from build123d import *

# Parameters (mm, degrees)
SKETCH1_R             = 162.5
SKETCH1_R_2           = 120
BOSS_EXTRUDE1_DEPTH   = 180
SKETCH2_R             = 135
CUT_EXTRUDE1_DEPTH    = 160
CHAMFER1_SIZE         = 1
CHAMFER1_SIZE2        = 3
CHAMFER2_SIZE         = 1
M8_TAPPED_HOLE1_D     = 6.8
M8_TAPPED_HOLE1_DEPTH = 26
M8_TAPPED_HOLE1_TIP   = 2.042926105


with BuildPart() as part:
    # Sketch1 → Boss-Extrude1 (new body)
    with BuildSketch(Plane(origin=(0, 0, 0), x_dir=(1, 0, 0), z_dir=(0, 1, 0))):
        with Locations(Location((0, 0, 0), (0, 0, 90))):
            Circle(SKETCH1_R)
        with Locations(Location((0, 0, 0), (0, 0, 90))):
            Circle(SKETCH1_R_2, mode=Mode.SUBTRACT)
    extrude(amount=BOSS_EXTRUDE1_DEPTH)

    # Sketch2 → Cut-Extrude1 (cut)
    with BuildSketch(Plane(origin=(0, 180, 0), x_dir=(1, 0, 0), z_dir=(0, 1, 0))):
        with Locations(Location((0, 0, 0), (0, 0, 270))):
            Circle(SKETCH2_R)
    extrude(amount=-CUT_EXTRUDE1_DEPTH, mode=Mode.SUBTRACT)

    # Chamfer1
    chamfer1_edges = [part.edges().sort_by_distance(p)[0] for p in [
        (0, 180, -135),
    ]]
    chamfer1_side = [part.faces().sort_by_distance(p)[0] for p in [
        (0, 180, 157.903805922),
    ]]
    chamfer(chamfer1_edges, length=CHAMFER1_SIZE, length2=CHAMFER1_SIZE2, reference=chamfer1_side[0])

    # Chamfer2
    chamfer2_edges = [part.edges().sort_by_distance(p)[0] for p in [
        (0, 20, 120),
        (0, 0, 120),
    ]]
    chamfer(chamfer2_edges, length=CHAMFER2_SIZE)

    # M8 Tapped Hole1
    with Locations(Plane(origin=(0, 180, 0), x_dir=(1, 0, 0), z_dir=(0, 1, 0))):
        with Locations((148, 0), (0, -148), (-148, 0), (0, 148)):
            Hole(M8_TAPPED_HOLE1_D / 2, depth=M8_TAPPED_HOLE1_DEPTH)
            with Locations((0, 0, -(M8_TAPPED_HOLE1_DEPTH + M8_TAPPED_HOLE1_TIP / 2))):  # 118° drill point
                Cone(0, M8_TAPPED_HOLE1_D / 2, M8_TAPPED_HOLE1_TIP, mode=Mode.SUBTRACT)


solid = part.part
Could you check a few things on this model? Use its own coordinates, in mm. A direction names the side the tool comes from. Coordinates: 2 decimals unless noted, no trailing zeros. Order: outer loops, then holes, each group sorted by start corner. A loop starts at its lowest first (then second) coordinate and runs counter-clockwise, first axis right, second up. Notation, with made-up numbers: (79, -1) -> (83, -1) arc R18 ccw to (83, 4) -> close; hole circle Ø10 at (-18, -36.75). An arc over 180 degrees is marked (long way). One line per item, written item: value. Start each with the question number.
1) We'd pull the mould along Z, two halves only. Please class faces 3 (the cylindrical face through (-137.02, 88.74, -87.36)), 4 (the cylindrical face through (-119.77, 99.6, 62.29)), 5 (the flat face through (84, 180, -108)): +Z half, -Z half, draft (parallel to the pull), parting line (faces both ways), or undercut.
2) If I drill on L1, parallel to X at y = 108, z = 0; L2, parallel to X at y = 153.5, z = 4.5; L3, parallel to Z at x = -148, y = 173, over which ranges is the centre line in solid material (lowest first)? Write a range as [from, to].
3) Which directions (+Z, -Z, +X, -X, +Y, -Y) give clear straight access to the entire face, cutting with the end or side of a thin tool? Please do faces 1 (the cylindrical face through (-5.276, 9.874, 119.884)), 2 (the flat face through (111, 20, -51)).
4) Imagine slicing it at B-B on y = 72.5. List the corners of the cut face in (x, z) for me, plus the area to 3 significant figures.
5) Imagine slicing it at A-A on y = 13.5. List the corners of the cut face in (x, z) for me, plus the area to 3 significant figures.
6) I'm going to push flat-ended pins straight in: pin 1 (6 mm diameter, centred on x = 104.5, y = 122.5, fed in from -Z); pin 2 (2 mm diameter, centred on y = 128, z = 70.5, fed in from -X); pin 3 (5 mm diameter, centred on x = -117.5, y = 42.5, fed in from -Z). Where does each tip first touch, or does it pass through?
Answer list:
1. face 3: parting line
1. face 4: undercut
1. face 5: draft
2. L1: x = [-162.5, -135], [135, 162.5]
2. L2: x = [-162.44, -134.92], [134.92, 162.44]
2. L3: z = [-67.1, -3.4], [3.4, 67.1]
3. face 1: +Y, -Y
3. face 2: +Y
4. outline: circle Ø325 at (0, 0); hole circle Ø270 at (0, 0)
4. area: 25,700 mm2
5. outline: circle Ø325 at (0, 0); hole circle Ø240 at (0, 0)
5. area: 37,700 mm2
6. pin 1: stops at z = -126.9
6. pin 2: stops at x = -146.89
6. pin 3: stops at z = -114.81
